Source: CAD feature listing. Evaluate the final solid. Frame: model axes, mm. Round coordinates to 2 decimals unless told otherwise and drop trailing zeros. Loops run counter-clockwise (first coordinate to the right, second up) from the corner with the lowest first, then second, coordinate; pieces in that order, holes last. Notation, with made-up numbers: (89, 88) -> (129, 88) arc R20 ccw to (129, 122) -> close; hole circle Ø9 at (60.5, -27.5). An arc over 180 degrees is marked (long way). Put each result on its own line as item: value. Start each with the question number.
1. Cut plane A-A (y = 11.05). Return the cut outline in (x, z), then the cut area to 3 significant figures.
2. Material intervals for L1, parallel to Z at x = 0.4, y = 3; L2, parallel to Y at x = 1.1, z = -13.5; L3, parallel to Z at x = 1.1, y = -35, sorted ascending.
3. Contact query for a flat-ended pin moving along its axis: pin 1 (3 mm diameter, centred on y = -29.75, z = -8, fed in from +X). Output: stop coordinate, or through.
4. Cut plane C-C (z = 14.5). Return the cut outline in (x, y).
5. Cut plane B-B (x = 0.4). State how many separate pieces and enclosed holes the cut face has, then the cut area to 3 significant figures.
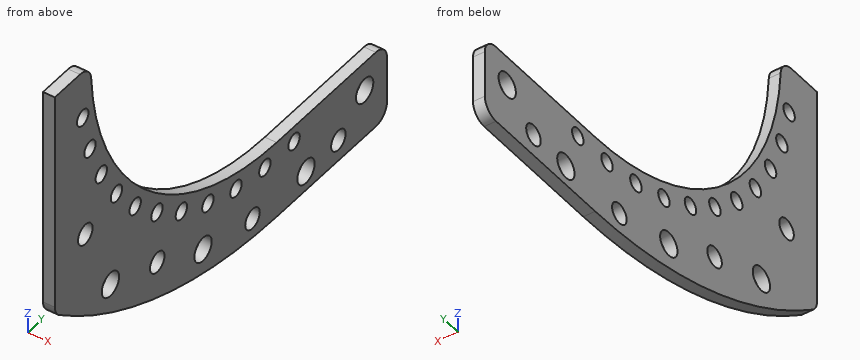
```python
from build123d import *

# Parameters (mm, degrees)
SKETCH_1_R      = 1.55
SKETCH_1_R_2    = 1.025
SKETCH_1_R_3    = 1.3
EXTRUDE_1_DEPTH = 1.5
FILLET_R2_1_R   = 2


with BuildPart() as part:
    # 草图1 → 凸台-拉伸1 (new body)
    with BuildSketch(Plane(origin=(0, 0, 0), x_dir=(0, 0, -1), z_dir=(1, 0, 0))):
        with BuildLine():
            Line((9.25, 19.75), (9.25, 0))
            ThreePointArc((9.25, 0), (-0.488699526, -23.511300474), (-24, -33.25))
            Line((-24, -33.25), (-24, -39.7))
            Line((-24, -39.7), (5.238932767, -39.7))
            ThreePointArc((5.238932767, -39.7), (15.644467461, -21.049940647), (19.25, 0))
            Line((19.25, 0), (19.25, 19.75))
            Line((19.25, 19.75), (9.25, 19.75))
        make_face()
        with Locations((13, 15.75)):
            Circle(SKETCH_1_R, mode=Mode.SUBTRACT)
        with Locations((11.25, 3.116215025)):
            Circle(SKETCH_1_R_2, mode=Mode.SUBTRACT)
        with Locations((-17.835585997, -34.70680769)):
            Circle(SKETCH_1_R_2, mode=Mode.SUBTRACT)
        with Locations((-12.773303956, -33.414424968)):
            Circle(SKETCH_1_R_2, mode=Mode.SUBTRACT)
        with Locations((-7.957653042, -31.387985027)):
            Circle(SKETCH_1_R_2, mode=Mode.SUBTRACT)
        with Locations((-3.494424789, -28.672005254)):
            Circle(SKETCH_1_R_2, mode=Mode.SUBTRACT)
        with Locations((0.518331383, -25.326151034)):
            Circle(SKETCH_1_R_2, mode=Mode.SUBTRACT)
        with Locations((3.992462152, -21.423925006)):
            Circle(SKETCH_1_R_2, mode=Mode.SUBTRACT)
        with Locations((6.851646862, -17.05105234)):
            Circle(SKETCH_1_R_2, mode=Mode.SUBTRACT)
        with Locations((9.033074163, -12.303597496)):
            Circle(SKETCH_1_R_2, mode=Mode.SUBTRACT)
        with Locations((10.488821863, -7.285853861)):
            Circle(SKETCH_1_R_2, mode=Mode.SUBTRACT)
        with Locations((11.1869097, -2.108052596)):
            Circle(SKETCH_1_R_2, mode=Mode.SUBTRACT)
        with Locations((16.57025586, -4.32369512)):
            Circle(SKETCH_1_R_3, mode=Mode.SUBTRACT)
        with Locations((14.615659071, -13.170834237)):
            Circle(SKETCH_1_R, mode=Mode.SUBTRACT)
        with Locations((16.5, 11.05)):
            Circle(SKETCH_1_R_3, mode=Mode.SUBTRACT)
        with Locations((16.75, 5.25)):
            Circle(SKETCH_1_R, mode=Mode.SUBTRACT)
        with Locations((-1.828452918, -34.25)):
            Circle(SKETCH_1_R_3, mode=Mode.SUBTRACT)
        with Locations((8, -29.75)):
            Circle(SKETCH_1_R, mode=Mode.SUBTRACT)
        with Locations((10.756717193, -21.368448937)):
            Circle(SKETCH_1_R_3, mode=Mode.SUBTRACT)
    extrude(amount=EXTRUDE_1_DEPTH)

    # R2 圆角1
    fillet_r2_1_edges = [part.edges().sort_by_distance(p)[0] for p in [
        (0.75, 19.75, -19.25),
        (0.75, -39.7, -5.238932767),
        (0.75, -33.25, 24),
        (0.75, 19.75, -9.25),
    ]]
    fillet(fillet_r2_1_edges, radius=FILLET_R2_1_R)


solid = part.part
```
Solution:
1. outline: (0, -19.25) -> (1.5, -19.25) -> (1.5, -17.8) -> (0, -17.8) -> close; (0, -15.2) -> (1.5, -15.2) -> (1.5, -9.25) -> (0, -9.25) -> close
1. area: 11.1 mm^2
2. L1: z = -19.25 to -12.27, -10.23 to -9.25
2. L2: y = -26.35 to -14.25, -12.09 to 14.28, 17.22 to 19.75
2. L3: z = -8.68 to 0.77, 2.89 to 16.85, 18.82 to 23.99
3. pin 1: passes through
4. outline: (0, -39.7) -> (1.5, -39.7) -> (1.5, -31.86) -> (0, -31.86) -> close
5. separate pieces: 1
5. enclosed holes: 19
5. area: 780 mm^2
